from build123d import *

# Parameters (mm, degrees)
BOSS_EXTRUDE1_DEPTH = 15
SKETCH2_R           = 3
CUT_EXTRUDE1_DEPTH  = 131.862523283


with BuildPart() as part:
    # Sketch1 → Boss-Extrude1 (new body)
    with BuildSketch(Plane.XY):
        Polygon((-3, 0), (-3, 65), (3, 65), (3, 0), (8, 0), (8, 65), (25, 65), (25, 120), (20, 120), (20, 70), (-20, 70), (-20, 120), (-25, 120), (-25, 65), (-8, 65), (-8, 0), align=None)
    extrude(amount=BOSS_EXTRUDE1_DEPTH)

    # Sketch2 → Cut-Extrude1 (cut, through all)
    with BuildSketch(Plane.ZY.offset(25)):
        with Locations(Location((7.5, 112.271855303, 0), (0, 0, 270))):
            Circle(SKETCH2_R)
        with Locations(Location((7.5, 12.271855303, 0), (0, 0, 270))):
            Circle(SKETCH2_R)
        with BuildLine():
            Line((0, 112.271855303), (-22.426817963, 115.88465347))
            Line((-22.426817963, 115.88465347), (0, 149.126440397))
            Line((0, 149.126440397), (35.619754134, 129.721336353))
            Line((35.619754134, 129.721336353), (15, 112.271855303))
            ThreePointArc((15, 112.271855303), (7.5, 119.771855303), (0, 112.271855303))
        make_face()
        with BuildLine():
            Line((0, 12.271855303), (-15.301630232, 4.771855303))
            Line((-15.301630232, 4.771855303), (-3.280552195, -11.427643596))
            Line((-3.280552195, -11.427643596), (32.469088575, -8.187179082))
            Line((32.469088575, -8.187179082), (24.8383173, 8.521855303))
            Line((24.8383173, 8.521855303), (15, 12.271855303))
            ThreePointArc((15, 12.271855303), (7.5, 4.771855303), (0, 12.271855303))
        make_face()
    extrude(amount=-CUT_EXTRUDE1_DEPTH, mode=Mode.SUBTRACT)


solid = part.part
The model under review builds one solid part; all positions refer to its coordinate system, in mm. A direction names the side the tool comes from. Give positions to 0.01 mm unless a question says otherwise; leave off trailing zeros. Loops run counter-clockwise (first coordinate to the right, second up) from the corner with the lowest first, then second, coordinate; pieces in that order, holes last. Notation, with made-up numbers: (80, 37.5) -> (125, 37.5) arc R17 cw to (125, 43.5) -> close; hole circle Ø10 at (45, 71.5). An arc over 180 degrees is marked (long way). Put each result on its own line as item: value. Start each with the question number.
1. We need section C-C on z = 12.5. State the section outline as (x, y) points.
2. Wall thickness on probe 1 along X at (y, z) = (18, 13.5); probe 2 along X at (y, z) = (104.5, 7); probe 3 along Y at (x, z) = (-15, 8.75): over which ranges is each line inside the solid? List them lowest first.
3. We need section A-A on z = 7.5. State how many separate pieces and enclosed holes the cut face has, then the cut area to 3 significant figures.
4. Clearance check with flat-ended pins moving along their axes: P1, Ø2, axis at x = -10, z = 9.5, coming from the -Y side; P2, Ø8, axis at y = 32, z = 11, coming from the -X side. State where each tip first meets the part, or that it passes through.
5. Mouldability with a two-part tool opening along X and no side actions: class faces 5 (the face through (-5.535, 4.774, 7.665)), 6 (the face through (0, 70, 7)), 7 (the face through (-8, 35, 7)) as released by +X, released by -X, zero draft, split by the parting line, or undercut.
6. We need section B-B on y = 59. State the section outline as (x, z) points.
7. For faces 1 (the face through (-17, 65, 7)), 2 (the face through (8, 34, 7)), 3 (the face through (20, 95, 7)), 4 (the face through (-3, 34, 7)), list the 3-axis set-ups (+Z, -Z, +X, -X, +Y, -Y) from which the entire face can be reached by the end or side of a thin tool; tool diameter is ignored.
8. We need section D-D on x = -18.5. State the section outline as (y, z) points, then the cut area to 3 significant figures.
Determined:
1. outline: (-25, 65) -> (-8, 65) -> (-8, 6.68) -> (-3, 6.68) -> (-3, 65) -> (3, 65) -> (3, 6.68) -> (8, 6.68) -> (8, 65) -> (25, 65) -> (25, 117.86) -> (20, 117.86) -> (20, 70) -> (-20, 70) -> (-20, 117.86) -> (-25, 117.86) -> close
2. probe 1: -8 to -3, 3 to 8
2. probe 2: -25 to -20, 20 to 25
2. probe 3: 65 to 70
3. separate pieces: 5
3. enclosed holes: 0
3. area: 1,230 mm^2
4. P1: y = 65
4. P2: x = -8
5. face 5: zero draft
5. face 6: undercut
5. face 7: released by -X
6. outline: (-8, 0) -> (-3, 0) -> (-3, 15) -> (-8, 15) -> close; (3, 0) -> (8, 0) -> (8, 15) -> (3, 15) -> close
7. face 1: +Z, -Z, -X, -Y
7. face 2: +Z, -Z, +X, -Y
7. face 3: +Z, -Z, +Y
7. face 4: +Z, -Z, -Y
8. outline: (65, 0) -> (70, 0) -> (70, 15) -> (65, 15) -> close
8. area: 75.0 mm^2
